Here's how the part is built. I have some questions about the finished solid (model axes, mm). A direction names the side the tool comes from. Coordinates: 2 decimals unless noted, no trailing zeros. Write each loop counter-clockwise with the first axis right and the second up, starting at its lowest first coordinate (ties: lowest second). Pieces come first, ordered by that corner, then holes.
```python
from build123d import *

# Parameters (mm, degrees)
SKETCH1_W           = 50
SKETCH1_H           = 50
SKETCH1_W_2         = 46
SKETCH1_H_2         = 46
BOSS_EXTRUDE1_DEPTH = 700
SKETCH2_R           = 7
CUT_EXTRUDE1_DEPTH  = 703.228595259


with BuildPart() as part:
    # Sketch1 → Boss-Extrude1 (new body)
    with BuildSketch(Plane.XY):
        Rectangle(SKETCH1_W, SKETCH1_H)
        Rectangle(SKETCH1_W_2, SKETCH1_H_2, mode=Mode.SUBTRACT)
    extrude(amount=BOSS_EXTRUDE1_DEPTH)

    # Sketch2 → Cut-Extrude1 (cut, through all)
    with BuildSketch(Plane.ZY.offset(25)):
        with Locations((289.5, 0)):
            Circle(SKETCH2_R)
        with Locations(Location((410.5, 0, 0), (0, 0, 180))):
            Circle(SKETCH2_R)
    extrude(amount=-CUT_EXTRUDE1_DEPTH, mode=Mode.SUBTRACT)


solid = part.part
```
1) Imagine slicing it at A-A on y = 0. Please give me the cut outline in (x, z), then the cut area to 3 significant figures.
Values follow:
outline: (-25, 0) - (-23, 0) - (-23, 282.5) - (-25, 282.5) - close; (-25, 296.5) - (-23, 296.5) - (-23, 403.5) - (-25, 403.5) - close; (-25, 417.5) - (-23, 417.5) - (-23, 700) - (-25, 700) - close; (23, 0) - (25, 0) - (25, 282.5) - (23, 282.5) - close; (23, 296.5) - (25, 296.5) - (25, 403.5) - (23, 403.5) - close; (23, 417.5) - (25, 417.5) - (25, 700) - (23, 700) - close
area: 2,690 mm2
2) Imagine slicing it at B-B on z = 272. Please give me the cut outline in (x, y).
Values follow:
outline: (-25, -25) - (25, -25) - (25, 25) - (-25, 25) - close; hole (-23, -23) - (23, -23) - (23, 23) - (-23, 23) - close
3) On a 3-axis mill with a long thin cutter (end or side, diameter ignored), from which of +Z, -Z, +X, -X, +Y, -Y can I reach the whole of each face in a straight line? I mean faces 1 (the face through (0, 23, 345)), 2 (the face through (0, -25, 345)). Say none if no direction works.
Values follow:
face 1: +Z, -Z
face 2: +Z, -Z, +X, -X, -Y
4) I need wall thicknesses on probe 1 along Y at (x, z) = (24.4, 410.5); probe 2 along Y at (x, z) = (14, 633.5). Which ranges of each line are inside material? Lowest first, please.
Values follow:
probe 1: y = -25 to -7, 7 to 25
probe 2: y = -25 to -23, 23 to 25
5) We'd pull the mould along Z, two halves only. Please class faces 3 (the face through (23.986, 2.103, 296.177)), 4 (the face through (-2, -24, 0)), 5 (the face through (23, 0, 345)): pulls with the +Z half, pulls with the -Z half, needs draft (parallel to the pull), parting line crosses it, or undercut.
Values follow:
face 3: undercut
face 4: pulls with the -Z half
face 5: needs draft
6) Will this pin go through, and if not, where does the flat tip stop? pin 1 (18 mm diameter, centred on y = 0, z = 289.5, fed in from +X).
Values follow:
pin 1: stops at x = 25
7) Imagine slicing it at C-C on x = 14.5. Please give me the cut outline in (y, z), then the cut area to 3 significant figures.
Values follow:
outline: (-25, 0) - (-23, 0) - (-23, 700) - (-25, 700) - close; (23, 0) - (25, 0) - (25, 700) - (23, 700) - close
area: 2,800 mm2
